Geometry check sheet. Reference: the model listing, model coordinates, mm. Give positions to 0.01 mm unless a question says otherwise; leave off trailing zeros. Write each loop counter-clockwise with the first axis right and the second up, starting at its lowest first coordinate (ties: lowest second). Pieces come first, ordered by that corner, then holes. Notation, with made-up numbers: (-31.75, -2) - (26.25, -2) arc R24 cw to (26.25, 29) - close; hole circle Ø7 at (63.25, 13.5). An arc over 180 degrees is marked (long way). Write item = value, one per line. Start each with the question number.
(1) Thickness scan on L1, parallel to X at y = -434, z = -26; L2, parallel to Y at x = 370, z = -26.25; L3, parallel to Z at x = 273.5, y = -329. Record the ranges inside material, lowest first.
(2) Section check B-B, the plane x = -318. Enter the section's corners in (y, z), plus the area to 3 significant figures.
(3) Depth check by flat-ended pin: pin 1 Ø4 at (x, y) = (-499.5, -77) entering from -Z. Enter the tip coordinate at first touch or a pass-through.
(4) Section check A-A, the plane y = -61. Enter the section's corners in (x, z), plus the area to 3 significant figures.
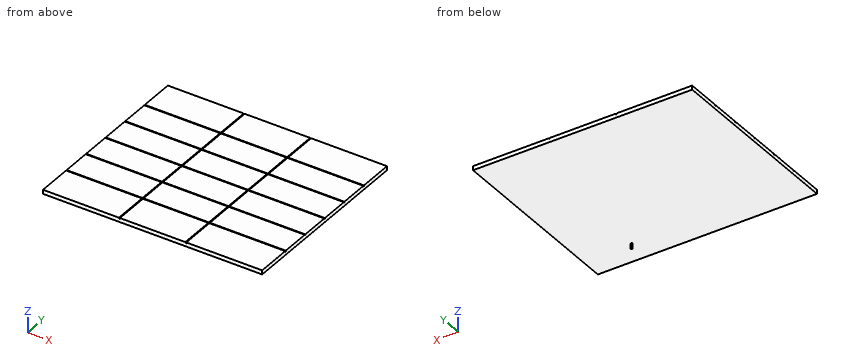
```python
from build123d import *

# Parameters (mm, degrees)
SKETCH1_W           = 1340
SKETCH1_H           = 1150
BOSS_EXTRUDE1_DEPTH = 25
SKETCH2_W           = 1379.704401218
SKETCH2_H           = 5
CUT_EXTRUDE1_DEPTH  = 5
SKETCH3_W           = 6
SKETCH3_H           = 1155.334708323
CUT_EXTRUDE2_DEPTH  = 5
LPATTERN1_COUNT     = 3
LPATTERN1_PITCH     = 180
LPATTERN1_COL_COUNT = 3
LPATTERN1_COL_PITCH = 180
SWEEP1_PROFILE_R    = 5
SKETCH13_R          = 1.5
CUT_EXTRUDE3_DEPTH  = 10


with BuildPart() as part:
    # Sketch1 → Boss-Extrude1 (new body)
    with BuildSketch(Plane.XY):
        Rectangle(SKETCH1_W, SKETCH1_H)
    extrude(amount=BOSS_EXTRUDE1_DEPTH)

    # Sketch2 → Cut-Extrude1 (cut)
    with BuildSketch(Plane.XY.offset(25)):
        Rectangle(SKETCH2_W, SKETCH2_H)
    cut_extrude1 = extrude(amount=-CUT_EXTRUDE1_DEPTH, mode=Mode.SUBTRACT)

    # Sketch3 → Cut-Extrude2 (cut)
    with BuildSketch(Plane.XY.offset(25)):
        with Locations((203, -0.575515136)):
            Rectangle(SKETCH3_W, SKETCH3_H)
        with Locations((-203, -0.575515136)):
            Rectangle(SKETCH3_W, SKETCH3_H)
    extrude(amount=-CUT_EXTRUDE2_DEPTH, mode=Mode.SUBTRACT)

    # LPattern1: Cut-Extrude1 ×3
    with Locations(*[(0, -i * LPATTERN1_PITCH, 0) for i in range(1, LPATTERN1_COUNT)]):
        add(cut_extrude1, mode=Mode.SUBTRACT)

    # LPattern1 col: Cut-Extrude1 ×3
    with Locations(*[(0, i * LPATTERN1_COL_PITCH, 0) for i in range(1, LPATTERN1_COL_COUNT)]):
        add(cut_extrude1, mode=Mode.SUBTRACT)

    # Sweep1: sweep along a path in Sketch4
    with BuildLine(Plane(origin=(-49.523696958, -434, -370.281312655), x_dir=(0.9899494936611666, 0, -0.14142135623730917), z_dir=(0, -1, 0))) as sweep1_path:
        Line((362.941585957, 425.889408172), (367.184226644, 396.190923362))
    # Sweep1 profile (on start of the path) → Sweep1 (sweep)
    with BuildSketch(Plane(origin=(370, -434, 0), x_dir=(-1, 0, 0), z_dir=(0, 0, -1))):
        Circle(SWEEP1_PROFILE_R)
    sweep(path=sweep1_path.line)

    # Sketch13 → Cut-Extrude3 (cut)
    with BuildSketch(Plane(origin=(0, 0, -30), x_dir=(-1, 0, 0), z_dir=(0, 0, -1))):
        with Locations((-370, -434)):
            Circle(SKETCH13_R)
    extrude(amount=-CUT_EXTRUDE3_DEPTH, mode=Mode.SUBTRACT)


solid = part.part
```
Model answer:
q1.L1 = 365 to 368.5, 371.5 to 375
q1.L2 = -439 to -435.5, -432.5 to -429
q1.L3 = 0 to 25
q2.outline = (-575, 0) - (575, 0) - (575, 25) - (362.5, 25) - (362.5, 20) - (357.5, 20) - (357.5, 25) - (182.5, 25) - (182.5, 20) - (177.5, 20) - (177.5, 25) - (2.5, 25) - (2.5, 20) - (-2.5, 20) - (-2.5, 25) - (-177.5, 25) - (-177.5, 20) - (-182.5, 20) - (-182.5, 25) - (-357.5, 25) - (-357.5, 20) - (-362.5, 20) - (-362.5, 25) - (-575, 25) - close
q2.area = 28,600 mm²
q3.pin_1 = 0
q4.outline = (-670, 0) - (670, 0) - (670, 25) - (206, 25) - (206, 20) - (200, 20) - (200, 25) - (-200, 25) - (-200, 20) - (-206, 20) - (-206, 25) - (-670, 25) - close
q4.area = 33,400 mm²
